from build123d import *

# Parameters (mm, degrees)
BASEHEAD_DEPTH     = 4
SKETCH6_R          = 4.35
CUT_EXTRUDE1_DEPTH = 1.4
CUT_EXTRUDE2_DEPTH = 0.572
CIRPATTERN2_COUNT  = 2
CIRPATTERN2_ANGLE  = 90


with BuildPart() as part:
    # Sketch2 → BaseHead (new body)
    with BuildSketch(Plane(origin=(0, 0, 0), x_dir=(0, 0, -1), z_dir=(1, 0, 0))):
        Polygon((2.886751346, -5), (5.773502692, 0), (2.886751346, 5), (-2.886751346, 5), (-5.773502692, 0), (-2.886751346, -5), align=None)
    extrude(amount=BASEHEAD_DEPTH)

    # Sketch10 → Revolve1 (revolve)
    with BuildSketch(Plane(origin=(0, 0, 0), x_dir=(1, 0, 0), z_dir=(0, 1, 0)), mode=Mode.PRIVATE) as revolve1_sk:
        with BuildLine():
            Line((4, 3.4), (4, 0))
            Line((4, 0), (39, 0))
            Line((39, 0), (39, 3))
            Line((39, 3), (7, 3))
            Line((7, 3), (5.507179677, 2.6))
            Line((5.507179677, 2.6), (4.8, 2.6))
            ThreePointArc((4.8, 2.6), (4.234314575, 2.834314575), (4, 3.4))
        make_face()
    revolve(revolve1_sk.sketch.rotate(Axis((0, 0, 0), (1, 0, 0)), 180), axis=Axis((0, 0, 0), (1, 0, 0)))

    # Sketch5 → HeadChamfer (revolve, cut)
    with BuildSketch(Plane(origin=(0, 0, 0), x_dir=(1, 0, 0), z_dir=(0, 1, 0)), mode=Mode.PRIVATE) as headchamfer_sk:
        Polygon((0, 5.773502692), (0.518112608, 5.773502692), (0, 4.35), align=None)
    revolve(headchamfer_sk.sketch.rotate(Axis((-0.358389262, 0, 0), (1, 0, 0)), 180), axis=Axis((-0.358389262, 0, 0), (1, 0, 0)), mode=Mode.SUBTRACT)

    # Sketch6 → Cut-Extrude1 (cut)
    with BuildSketch(Plane.ZY):
        Circle(SKETCH6_R)
    extrude(amount=-CUT_EXTRUDE1_DEPTH, mode=Mode.SUBTRACT)

    # Sketch7 → Cut-Extrude2 (cut, symmetric)
    with BuildSketch(Plane(origin=(0, 0, 0), x_dir=(1, 0, 0), z_dir=(0, 1, 0))):
        Polygon((4.26, 0), (0.9, 3.641958042), (0.9, -3.641958042), align=None)
    cut_extrude2 = extrude(amount=CUT_EXTRUDE2_DEPTH, both=True, mode=Mode.SUBTRACT)

    # CirPattern2: Cut-Extrude2 ×2 about axis
    cirpattern2_axis = Axis((0, 0, 0), (-1, 0, 0))
    for i in range(1, CIRPATTERN2_COUNT):
        add(cut_extrude2.rotate(cirpattern2_axis, i * CIRPATTERN2_ANGLE / (CIRPATTERN2_COUNT - 1)), mode=Mode.SUBTRACT)


solid = part.part
Read the model definition and answer for the solid it produces. Units are mm, in the model's axes. A direction names the side the tool comes from. Coordinates: 2 decimals unless noted, no trailing zeros. Loops run counter-clockwise (first coordinate to the right, second up) from the corner with the lowest first, then second, coordinate; pieces in that order, holes last. Notation, with made-up numbers: (11.5, 13.5) - (19.5, 13.5) arc R20 cw to (19.5, 21.5) - close; hole circle Ø6 at (8, 0). An arc over 180 degrees is marked (long way). Answer in a Markdown table with one row per item.
Q1. For faces 4 (the flat face through (4, 3.4, -1.2)), 5 (the flat face through (2, 0.572, 2)), 6 (the flat face through (2.092, 2.535, 4.31)), determine the directions among +Z, -Z, +X, -X, +Y, -Y from which every point of the face is accessible in a straight line to the end or side of a thin tool.
Here are the results:
| item | result |
|---|---|
| face 4 | +X |
| face 5 | -X |
| face 6 | +Z, +X, -X, +Y |
Q2. The mould has two halves that part along Y. Classify faces 1 (the cylindrical face through (22.78, -0.9, 2.86)), 2 (the cylindrical face through (0.69, -4.247, -0.943)), 3 (the flat face through (2.092, -2.535, -4.31)): pulls with the +Y half, pulls with the -Y half, needs draft (parallel to the pull), parting line crosses it, or undercut.
Here are the results:
| item | result |
|---|---|
| face 1 | parting line crosses it |
| face 2 | undercut |
| face 3 | pulls with the -Y half |
Q3. Find section A-A on x = 29. Write down the section's boundary in (y, z), plus the area to 3 significant figures.
Here are the results:
| item | result |
|---|---|
| outline | circle Ø6 at (0, 0) |
| area | 28.3 mm^2 |
Q4. Given P1, Ø3, axis at y = -2, z = -2.5, coming from the +X side; P2, Ø3, axis at x = 8.5, y = 3, coming from the +Z side; P3, Ø1.2, axis at x = 2.5, y = 2, coming from the -Z side; P4, Ø1, axis at y = -3.5, z = 1.5, coming from the +X side, each flat-ended and moving along its own axis, determine where each tip first touches the part or whether it passes through.
Here are the results:
| item | result |
|---|---|
| P1 | stops at x = 39 |
| P2 | stops at z = 2.6 |
| P3 | stops at z = -4.97 |
| P4 | stops at x = 4.01 |
Q5. Straight lines are drawn through the part: line 1 along Y through (x, z) = (0.65, 0); line 2 along X through (y, z) = (1.75, -3.75); line 3 along Y through (x, z) = (17.5, 0). For each, find the intervals that lie inside material, in ascending order. Write a range as [from, to].
Here are the results:
| item | result |
|---|---|
| line 1 | y = [-5, -4.35], [4.35, 5] |
| line 2 | x = [1.4, 4] |
| line 3 | y = [-3, 3] |
